Design review of the part built by this model. Coordinates are the model's own, in mm. A direction names the side the tool comes from. Round coordinates to 2 decimals unless told otherwise and drop trailing zeros. Write each loop counter-clockwise with the first axis right and the second up, starting at its lowest first coordinate (ties: lowest second). Pieces come first, ordered by that corner, then holes. Notation, with made-up numbers: (-15.5, 38) -> (8.5, 38) arc R13 cw to (8.5, 61) -> close; hole circle Ø4 at (45, -1). An arc over 180 degrees is marked (long way). One line per question, with ' | ' between items. Start each with the question number.
1) Insertion check: pin 1 Ø2 at (y, z) = (49, 6.5) entering from -X; pin 2 Ø1 at (x, z) = (206, -29) entering from -Y; pin 3 Ø2 at (y, z) = (64.5, -2) entering from -X. Each pin has a flat end and moves straight along its axis. Give the tip position at first contact, or say it passes through.
2) Consider section B-B (z = -37). Give the boundary of the cut face in (x, y), then the cut area to 3 significant figures.
3) For faces 1 (the flat face through (213.34, 99.95, -42.41)), 2 (the cylindrical face through (79.493, 26.325, 7.437)), 3 (the cylindrical face through (208.495, 73.716, -21.166)), list the 3-axis set-ups (+Z, -Z, +X, -X, +Y, -Y) from which the entire face can be reached by the end or side of a thin tool; tool diameter is ignored.
4) For probe 1 along Z at (x, y) = (94.5, 24); probe 2 along Y at (x, z) = (28, 9); probe 3 along Z at (x, y) = (231, 71.5), list the stretches that pass through material, from the lowest coordinate up.
5) Consider section A-A (z = 6). Give the boundary of the cut face in (x, y), then the cut area to 3 significant figures.
6) Mouldability with a two-part tool opening along Z and no side actions: class faces 4 (the flat face through (93, 19, 15)), 5 (the flat face through (232.79, 64.99, -42.41)), 6 (the flat face through (93, 19, 0)), 7 (the flat face through (227, 85, -1.566)) as +Z half, -Z half, draft (parallel to the pull), parting line (faces both ways), or undercut.
```python
from build123d import *

# Parameters (mm, degrees)
BOSS_EXTRUDE1_DEPTH      = 15
FILLET1_R                = 3
SKETCH2_R                = 15
CUT_EXTRUDE1_DEPTH       = 253.670657786
BOSS_EXTRUDE2_DEPTH      = 45
BOSS_EXTRUDE2_DEPTH_BACK = 17
SKETCH6_W                = 83.616638364
SKETCH6_H                = 38.333633137
CUT_EXTRUDE3_DEPTH       = 289.058075248
SKETCH8_R                = 2.5
BOSS_EXTRUDE3_DEPTH      = 38
LPATTERN1_COUNT          = 3
LPATTERN1_PITCH          = 20


with BuildPart() as part:
    # Sketch1 → Boss-Extrude1 (new body)
    with BuildSketch(Plane.XY):
        with BuildLine():
            Line((0, 25), (69.282032303, 25))
            ThreePointArc((69.282032303, 25), (79.634794107, 26.362966948), (89.282032303, 30.358983849))
            Line((89.282032303, 30.358983849), (209.903810568, 100))
            Line((209.903810568, 100), (231.554445662, 62.5))
            Line((231.554445662, 62.5), (89.282032303, -19.641016151))
            ThreePointArc((89.282032303, -19.641016151), (79.634794107, -23.637033052), (69.282032303, -25))
            Line((69.282032303, -25), (0, -25))
            ThreePointArc((0, -25), (-25, 0), (0, 25))
        make_face()
    extrude(amount=BOSS_EXTRUDE1_DEPTH)

    # Fillet1
    fillet1_edges = [part.edges().sort_by_distance(p)[0] for p in [
        (160.418238983, 21.429491924, 0),
        (79.634794107, -23.637033052, 0),
        (34.641016151, -25, 0),
        (-25, 0, 0),
        (79.634794107, -23.637033052, 15),
        (160.418238983, 21.429491924, 15),
        (149.592921435, 65.179491924, 15),
        (79.634794107, 26.362966948, 15),
        (34.641016151, 25, 15),
        (-25, 0, 15),
        (34.641016151, 25, 0),
        (34.641016151, -25, 15),
        (79.634794107, 26.362966948, 0),
        (149.592921435, 65.179491924, 0),
        (220.729128115, 81.25, 0),
    ]]
    fillet(fillet1_edges, radius=FILLET1_R)

    # Sketch2 → Cut-Extrude1 (cut, through all)
    with BuildSketch(Plane.XY.offset(15)):
        Circle(SKETCH2_R)
    extrude(amount=-CUT_EXTRUDE1_DEPTH, mode=Mode.SUBTRACT)

    # Sketch3 → Boss-Extrude2 (add, two sides: drawn at the far end of the back side and taken through both)
    with BuildSketch(Plane(origin=(0, 0, 0), x_dir=(-1, 0, 0), z_dir=(0, 0, -1)).offset(-BOSS_EXTRUDE2_DEPTH_BACK)):
        with BuildLine():
            Line((-232.55316524, 111.042650187), (-193.582022069, 88.542650187))
            ThreePointArc((-193.582022069, 88.542650187), (-186.261513994, 61.222142112), (-213.582022069, 53.901634036))
            Line((-213.582022069, 53.901634036), (-252.55316524, 76.401634036))
            ThreePointArc((-252.55316524, 76.401634036), (-259.873673315, 103.722142112), (-232.55316524, 111.042650187))
        make_face()
    extrude(amount=BOSS_EXTRUDE2_DEPTH + BOSS_EXTRUDE2_DEPTH_BACK)

    # Sketch6 → Cut-Extrude3 (cut, through all)
    with BuildSketch(Plane(origin=(10.055413327, -17.416486774, 0), x_dir=(0.8660254037844389, 0.4999999999999995, 0), z_dir=(-0.4999999999999995, 0.8660254037844389, 0))):
        with Locations((244.569446826, 20.732918796)):
            Rectangle(SKETCH6_W, SKETCH6_H)
    extrude(amount=-CUT_EXTRUDE3_DEPTH, mode=Mode.SUBTRACT)

    # Sketch8 → Boss-Extrude3 (add)
    with BuildSketch(Plane.XY.offset(-39.899735364)):
        with Locations(Location((240.638883171, 93.826084401, 0), (0, 0, 180))):
            Circle(SKETCH8_R)
    boss_extrude3 = extrude(amount=BOSS_EXTRUDE3_DEPTH)

    # LPattern1: Boss-Extrude3 ×3
    with Locations(*[Vector(-0.8660254037844388, -0.49999999999999983, 0) * (i * LPATTERN1_PITCH) for i in range(1, LPATTERN1_COUNT)]):
        add(boss_extrude3)


solid = part.part
```
From the geometry:
1) pin 1: stops at x = 119.84 | pin 2: stops at y = 71.33 | pin 3: stops at x = 184.42
2) outline: (186.76, 82.04) arc R20 ccw to (204.54, 51.25) -> close; circle Ø5 at (206, 73.83); circle Ø5 at (223.32, 83.83); circle Ø5 at (240.64, 93.83) | area: 334 mm2
3) face 1: -Z, -X, +Y | face 2: +Z, -Z, -X, +Y | face 3: none
4) probe 1: z = 0 to 15 | probe 2: y = -25 to 25 | probe 3: z = -45 to -39.9, -1.57 to 17
5) outline: (0, -25) -> (69.28, -25) arc R40 ccw to (89.28, -19.64) -> (231.55, 62.5) -> (230.78, 63.83) -> (252.55, 76.4) arc R20 ccw to (232.55, 111.04) -> (210.78, 98.47) -> (209.9, 100) -> (89.28, 30.36) arc R40 cw to (69.28, 25) -> (0, 25) arc R25 ccw to start; hole circle Ø30 at (0, 0) | area: 12,900 mm2
6) face 4: +Z half | face 5: draft | face 6: -Z half | face 7: undercut
